Verification items for the finished model (mm, model axes). Face numbers are marked on the shaded views. Round coordinates to 2 decimals unless told otherwise and drop trailing zeros. Answer in a Markdown table with one row per item. Add a question column.
1. Draft check along Y on the marked faces 1, 2 and 3. Enter one of: pulls with the +Y half, pulls with the -Y half, needs draft (parallel to the pull), parting line crosses it, or undercut.
2. Go/stop test with flat-tipped pins: pin 1 Ø8 at (x, z) = (86.5, 25) entering from -Y; pin 2 Ø3 at (x, z) = (90, 4) entering from -Y; pin 3 Ø3 at (y, z) = (-100, 26.5) entering from -X. Record where each tip stops, or that it passes through.
3. Material ranges on probe 1 along Y at (x, z) = (95.5, 11); probe 2 along Y at (x, z) = (85, 20), recorded low to high.
```python
from build123d import *

# Parameters (mm, degrees)
SKETCH1_W           = 100
SKETCH1_H           = 335
BOSS_EXTRUDE1_DEPTH = 35
CHAMFER1_SIZE       = 20


with BuildPart() as part:
    # Sketch1 → Boss-Extrude1 (new body)
    with BuildSketch(Plane.XY):
        with Locations((50, -167.5)):
            Rectangle(SKETCH1_W, SKETCH1_H)
    extrude(amount=BOSS_EXTRUDE1_DEPTH)

    # Chamfer1
    chamfer1_edges = [part.edges().sort_by_distance(p)[0] for p in [
        (100, -335, 17.5),
    ]]
    chamfer(chamfer1_edges, length=CHAMFER1_SIZE)


solid = part.part
```
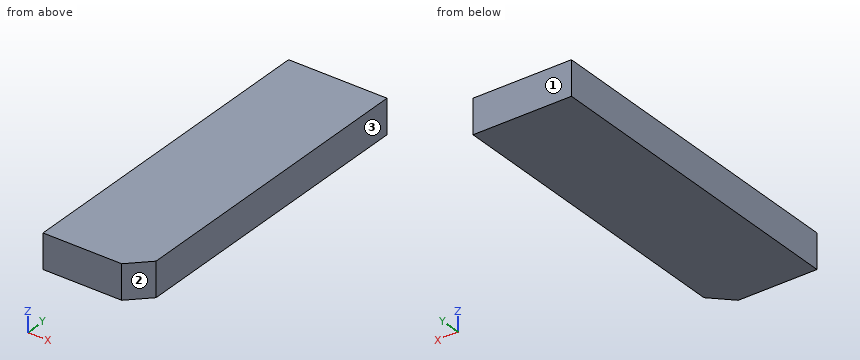
Geometry check:
| question | item | result |
|---|---|---|
| 1 | face 1 | pulls with the +Y half |
| 1 | face 2 | pulls with the -Y half |
| 1 | face 3 | needs draft |
| 2 | pin 1 | stops at y = -332.5 |
| 2 | pin 2 | stops at y = -326.5 |
| 2 | pin 3 | stops at x = 0 |
| 3 | probe 1 | y = -319.5 to 0 |
| 3 | probe 2 | y = -330 to 0 |
